from build123d import *

# Parameters (mm, degrees)
SKETCH1_W           = 98.4
SKETCH1_H           = 98.4
SKETCH1_R           = 2.55
BOSS_EXTRUDE1_DEPTH = 0.8


with BuildPart() as part:
    # Sketch1 → Boss-Extrude1 (new body)
    with BuildSketch(Plane(origin=(0, 0, 0), x_dir=(1, 0, 0), z_dir=(0, 1, 0))):
        Rectangle(SKETCH1_W, SKETCH1_H)
        with Locations(Location((0, 0, 0), (0, 0, 270))):
            Circle(SKETCH1_R, mode=Mode.SUBTRACT)
    extrude(amount=BOSS_EXTRUDE1_DEPTH)


solid = part.part
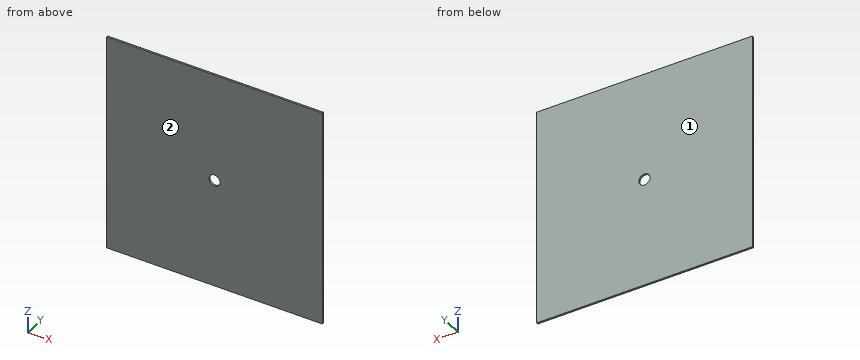
For this review, take the finished solid that the model builds, in its own axes (mm). Face numbers are marked on the shaded views. Give positions to 0.01 mm unless a question says otherwise; leave off trailing zeros. Loops run counter-clockwise (first coordinate to the right, second up) from the corner with the lowest first, then second, coordinate; pieces in that order, holes last. Notation, with made-up numbers: M -15.75,-15 L 28.25,-15 A32 cw 28.25,17 Z; hole C -6.5,24.25 d9. An arc over 180 degrees is marked long. Put each result on its own line as item: value. Start each with the question number.
(1) Add section B-B, the plane x = 0. Write out the cut boundary in (y, z).
(2) Wall thickness on L1, parallel to X at y = 0.3, z = 0; L2, parallel to Z at x = 2, y = 0.1: over which ranges is each line inside the solid? List them lowest first.
(3) The part is to be moulded in two halves that separate along Y. For the marked faces 1 and 2, say which applies: +Y half, -Y half, draft (parallel to the pull), parting line (faces both ways), or undercut.
(4) Add section A-A, the plane z = 0. Write out the cut boundary in (x, y).
Result:
1. outline: M 0,-49.2 L 0.8,-49.2 L 0.8,-2.55 L 0,-2.55 Z; M 0,2.55 L 0.8,2.55 L 0.8,49.2 L 0,49.2 Z
2. L1: x = -49.2 to -2.55, 2.55 to 49.2
2. L2: z = -49.2 to -1.58, 1.58 to 49.2
3. face 1: +Y half
3. face 2: -Y half
4. outline: M -49.2,0 L -2.55,0 L -2.55,0.8 L -49.2,0.8 Z; M 2.55,0 L 49.2,0 L 49.2,0.8 L 2.55,0.8 Z
